from build123d import *

# Parameters (mm, degrees)
SKETCH_1_W      = 35
SKETCH_1_H      = 100
EXTRUDE_1_DEPTH = 10
SKETCH_2_R      = 12.5
EXTRUDE_2_DEPTH = 30
SKETCH_3_R      = 9
EXTRUDE_3_DEPTH = 25


with BuildPart() as part:
    # 草图1 → 凸台-拉伸1 (new body)
    with BuildSketch(Plane.XY):
        Rectangle(SKETCH_1_W, SKETCH_1_H)
    extrude(amount=EXTRUDE_1_DEPTH)

    # 草图2 → 凸台-拉伸2 (add)
    with BuildSketch(Plane.XY.offset(10)):
        with Locations(Location((0, 30, 0), (0, 0, 180))):
            Circle(SKETCH_2_R)
    extrude(amount=EXTRUDE_2_DEPTH)

    # 草图3 → 凸台-拉伸3 (add)
    with BuildSketch(Plane(origin=(0, 0, 0), x_dir=(-1, 0, 0), z_dir=(0, 0, -1))):
        with Locations((0, 30)):
            Circle(SKETCH_3_R)
    extrude(amount=EXTRUDE_3_DEPTH)


solid = part.part
The listing builds one solid part. Answer for the finished solid, in the listing's coordinates (mm). A direction names the side the tool comes from. Give positions to 0.01 mm unless a question says otherwise; leave off trailing zeros. Write each loop counter-clockwise with the first axis right and the second up, starting at its lowest first coordinate (ties: lowest second). Pieces come first, ordered by that corner, then holes. Notation, with made-up numbers: (-37.75, -16.75) - (11.25, -16.75) arc R10 ccw to (11.25, 1.25) - close; hole circle Ø11 at (39.25, -25.5). An arc over 180 degrees is marked (long way). One line per question, with ' | ' between items. Start each with the question number.
1. Section A-A, the plane x = 0 is taken. Determine the outline of the cut face in (y, z), then the cut area to 3 significant figures.
2. Straight lines are drawn through the part: line 1 (Z direction, x = 10.5, y = -21); line 2 (Z direction, x = 6, y = 22.5); line 3 (X direction, y = 29, z = 18). For each, find the intervals that lie inside material, in ascending order.
3. Given P1, Ø4, axis at y = 23.5, z = -9, coming from the +X side; P2, Ø10.5, axis at x = -8, y = 14, coming from the +Z side; P3, Ø4, axis at x = 2, y = -38.5, coming from the -Z side, each flat-ended and moving along its own axis, determine where each tip first touches the part or whether it passes through.
4. Section C-C, the plane z = -16.5 is taken. Determine the outline of the cut face in (x, y), then the cut area to 3 significant figures.
5. Section B-B, the plane y = 30 is taken. Determine the outline of the cut face in (x, z).
6. Section D-D, the plane x = -10 is taken. Determine the outline of the cut face in (y, z).
7. For faces 1 (the face through (2.71, 42.203, 24.79)), 2 (the face through (-4.84, 37.59, -12.32)), 3 (the face through (-17.5, -1, 5)), determine the directions among +Z, -Z, +X, -X, +Y, -Y from which every point of the face is accessible in a straight line to the end or side of a thin tool.
Result:
1) outline: (-50, 0) - (21, 0) - (21, -25) - (39, -25) - (39, 0) - (50, 0) - (50, 10) - (42.5, 10) - (42.5, 40) - (17.5, 40) - (17.5, 10) - (-50, 10) - close | area: 2,200 mm2
2) line 1: z = 0 to 10 | line 2: z = 0 to 40 | line 3: x = -12.46 to 12.46
3) P1: stops at x = 7.79 | P2: stops at z = 10 | P3: stops at z = 0
4) outline: circle Ø18 at (0, 30) | area: 254 mm2
5) outline: (-17.5, 0) - (-9, 0) - (-9, -25) - (9, -25) - (9, 0) - (17.5, 0) - (17.5, 10) - (12.5, 10) - (12.5, 40) - (-12.5, 40) - (-12.5, 10) - (-17.5, 10) - close
6) outline: (-50, 0) - (50, 0) - (50, 10) - (37.5, 10) - (37.5, 40) - (22.5, 40) - (22.5, 10) - (-50, 10) - close
7) face 1: +Z | face 2: -Z | face 3: +Z, -Z, -X, +Y, -Y
